Design review of the part shown in the three views and the two pictorial views. Dimensions are in mm from the part's minimum x, y and z. A direction names the side the tool comes from. Give positions to 0.01 mm unless a question says otherwise; leave off trailing zeros. Order: outer loops, then holes, each group sorted by start corner. A loop starts at its lowest first (then second) coordinate and runs counter-clockwise, first axis right, second up. Notation, with made-up numbers: (10.25, -2.75) - (41.25, -2.75) arc R32 cw to (41.25, 26.25) - close; hole circle Ø8 at (81, 34.25). An arc over 180 degrees is marked (long way). Put each result on its own line as item: value.
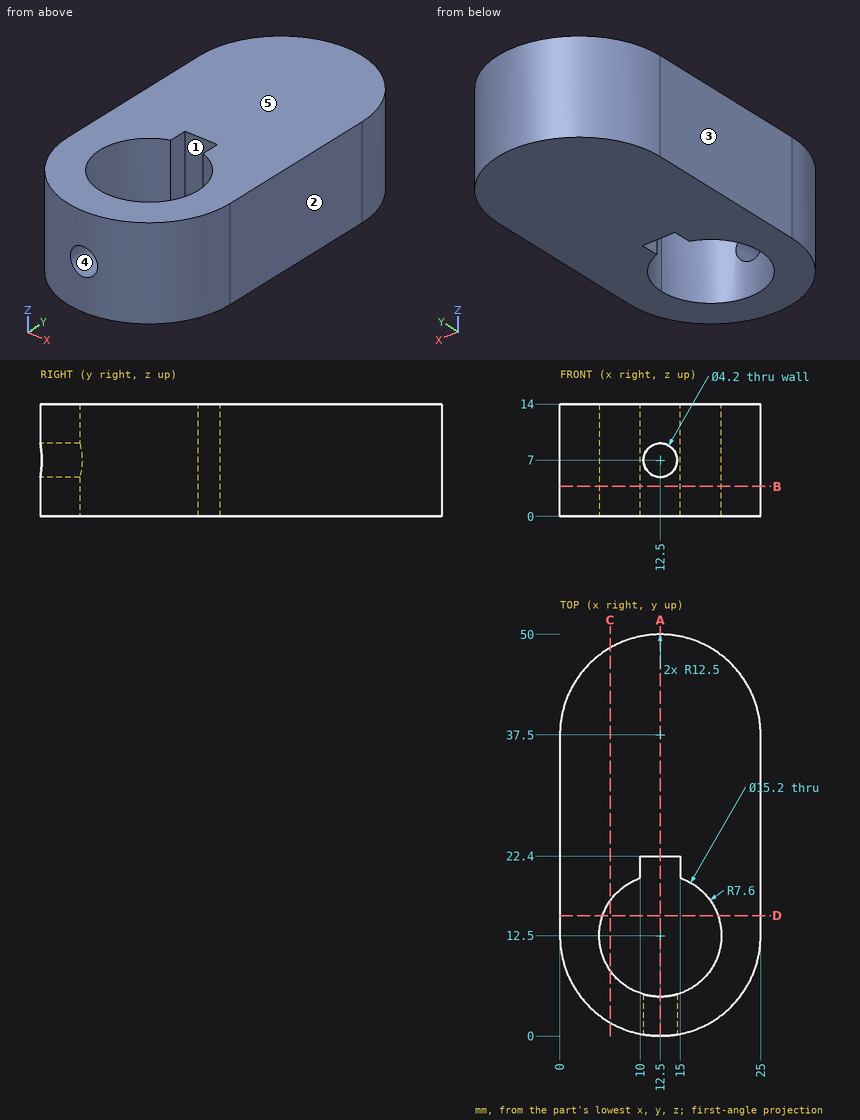
(1) The part is to be moulded in two halves that separate along Z. For the marked faces 3, 4 and 5, say which applies: pulls with the +Z half, pulls with the -Z half, needs draft (parallel to the pull), parting line crosses it, or undercut.
The answers:
face 3: needs draft
face 4: undercut
face 5: pulls with the +Z half
(2) Take a section at B-B, the plane z = 3.75. Write out the cut boundary in (x, y).
The answers:
outline: (0, 12.5) arc R12.5 ccw to (25, 12.5) - (25, 37.5) arc R12.5 ccw to (0, 37.5) - close; hole (10, 19.68) arc R7.6 ccw (long way) to (15, 19.68) - (15, 22.4) - (10, 22.4) - close
(3) Take a section at C-C, the plane x = 6.25. Write out the cut boundary in (y, z), then the cut area to 3 significant figures.
The answers:
outline: (1.67, 0) - (8.18, 0) - (8.18, 14) - (1.67, 14) - close; (16.82, 0) - (48.33, 0) - (48.33, 14) - (16.82, 14) - close
area: 532 mm^2
(4) Take a section at D-D, the plane y = 15. Write out the cut boundary in (x, z), then the cut area to 3 significant figures.
The answers:
outline: (0, 0) - (5.32, 0) - (5.32, 14) - (0, 14) - close; (19.68, 0) - (25, 0) - (25, 14) - (19.68, 14) - close
area: 149 mm^2
(5) Wall thickness on L1, parallel to X at y = 20, z = 10.5; L2, parallel to Y at x = 12.5, z = 5.75; L3, parallel to Y at x = 17.25, z = 11: over which ranges is each line inside the solid? List them lowest first.
The answers:
L1: 0 to 10, 15 to 25
L2: 22.4 to 50
L3: 0.94 to 6.57, 18.43 to 49.06
(6) Clearance check with flat-ended pins moving along their axes: pin 1 Ø13.5 at (x, y) = (12.5, 12.5) entering from +Z; pin 2 Ø5 at (x, z) = (6, 7.5) entering from +Y. State where each tip first meets the part, or that it passes through.
The answers:
pin 1: through
pin 2: y = 49.34
(7) Take a section at A-A, the plane x = 12.5. Write out the cut boundary in (y, z), then the cut area to 3 significant figures.
The answers:
outline: (0, 0) - (4.9, 0) - (4.9, 4.9) - (0, 4.9) - close; (0, 9.1) - (4.9, 9.1) - (4.9, 14) - (0, 14) - close; (22.4, 0) - (50, 0) - (50, 14) - (22.4, 14) - close
area: 434 mm^2
(8) For the marked faces 1 and 2, list the 3-axis set-ups (+Z, -Z, +X, -X, +Y, -Y) from which the entire face can be reached by the end or side of a thin tool; tool diameter is ignored.
The answers:
face 1: +Z, -Z
face 2: +Z, -Z, +X, +Y, -Y
